The listing builds one solid part. Answer for the finished solid, in the listing's coordinates (mm). Give positions to 0.01 mm unless a question says otherwise; leave off trailing zeros. Write each loop counter-clockwise with the first axis right and the second up, starting at its lowest first coordinate (ties: lowest second). Pieces come first, ordered by that corner, then holes. Notation, with made-up numbers: (-9.5, -25) - (43.5, -25) arc R19 ccw to (43.5, -3) - close; hole circle Ø9 at (-37, -17). An arc over 180 degrees is marked (long way). One line per question, with ' | ' between items. Start each with the question number.
1. A cutting plane is placed at C-C (y = 1.55). Determine the outline of the cut face in (x, z).
2. A cutting plane is placed at D-D (x = 124). Determine the outline of the cut face in (y, z).
3. A cutting plane is placed at A-A (z = -78). Determine the outline of the cut face in (x, y).
4. Find the intervals of material crossed by L1, parallel to X at y = 2.55, z = 17.5; L2, parallel to X at y = 2.65, z = -17.5; L3, parallel to X at y = 1.8, z = 14, in increasing order. Write a range as from..to.
5. Given P1, Ø4, axis at x = -130.89, z = -17.5, coming from the -Y side; P2, Ø0.9, axis at y = 1.5, z = -78, coming from the -X side; P3, Ø1, axis at x = -99, y = 1, coming from the +Z side, each flat-ended and moving along its own axis, determine where each tip first touches the part or whether it passes through.
6. A cutting plane is placed at B-B (x = 13). Determine the outline of the cut face in (y, z), then the cut area to 3 significant figures.
```python
from build123d import *

# Parameters (mm, degrees)
SKETCH1_R           = 142.5
BOSS_EXTRUDE1_DEPTH = 3
SKETCH3_R           = 11
CUT_EXTRUDE1_DEPTH  = 10
CIRPATTERN1_COUNT   = 3
CUT_EXTRUDE2_DEPTH  = 10
CUT_EXTRUDE3_DEPTH  = 10
CUT_EXTRUDE6_START  = -10
CUT_EXTRUDE6_DEPTH  = 10
FILLET1_R           = 3
SKETCH7_W           = 9
SKETCH7_H           = 120
CUT_EXTRUDE7_DEPTH  = 10
SKETCH8_R           = 1.75
CUT_EXTRUDE8_DEPTH  = 10
CHAMFER1_SIZE       = 2.2


with BuildPart() as part:
    # Sketch1 → Boss-Extrude1 (new body)
    with BuildSketch(Plane(origin=(0, 0, 0), x_dir=(1, 0, 0), z_dir=(0, 1, 0))):
        with Locations(Location((0, 0, 0), (0, 0, 270))):
            Circle(SKETCH1_R)
    extrude(amount=BOSS_EXTRUDE1_DEPTH)

    # Sketch3 → Cut-Extrude1 (cut)
    with BuildSketch(Plane(origin=(0, 3, 0), x_dir=(1, 0, 0), z_dir=(0, 1, 0))):
        with Locations(Location((0, -26.5, 0), (0, 0, 270))):
            Circle(SKETCH3_R)
    cut_extrude1 = extrude(amount=-CUT_EXTRUDE1_DEPTH, mode=Mode.SUBTRACT)

    # CirPattern1: Cut-Extrude1 ×3 about axis
    cirpattern1_axis = Axis((0, 0, 0), (0, 1, 0))
    for i in range(1, CIRPATTERN1_COUNT):
        add(cut_extrude1.rotate(cirpattern1_axis, i * 360 / CIRPATTERN1_COUNT), mode=Mode.SUBTRACT)

    # Sketch4 → Cut-Extrude2 (cut)
    with BuildSketch(Plane(origin=(0, 3, 0), x_dir=(1, 0, 0), z_dir=(0, 1, 0))):
        with BuildLine():
            Line((-32.475952642, 7.75), (-9.526279442, -32))
            ThreePointArc((-9.526279442, -32), (0, -37.5), (9.526279442, -32))
            Line((9.526279442, -32), (32.475952642, 7.75))
            ThreePointArc((32.475952642, 7.75), (32.475952642, 18.75), (22.9496732, 24.25))
            Line((22.9496732, 24.25), (-22.9496732, 24.25))
            ThreePointArc((-22.9496732, 24.25), (-32.475952642, 18.75), (-32.475952642, 7.75))
        make_face()
    extrude(amount=-CUT_EXTRUDE2_DEPTH, mode=Mode.SUBTRACT)

    # Sketch5 → Cut-Extrude3 (cut)
    with BuildSketch(Plane(origin=(0, 3, 0), x_dir=(1, 0, 0), z_dir=(0, 1, 0))):
        with BuildLine():
            Line((-5, 45), (-5, 95))
            ThreePointArc((-5, 95), (0, 100), (5, 95))
            Line((5, 95), (5, 45))
            ThreePointArc((5, 45), (0, 40), (-5, 45))
        make_face()
    extrude(amount=-CUT_EXTRUDE3_DEPTH, mode=Mode.SUBTRACT)

    # Sketch6 → Cut-Extrude6 (cut)
    with BuildSketch(Plane(origin=(0, 3, 0), x_dir=(1, 0, 0), z_dir=(0, 1, 0)).offset(CUT_EXTRUDE6_START)):
        with BuildLine():
            Line((89.596317401, -110.809520837), (82.482737092, -103.695940527))
            ThreePointArc((82.482737092, -103.695940527), (93.691648507, -93.691648507), (103.695940527, -82.482737092))
            Line((103.695940527, -82.482737092), (110.809520837, -89.596317401))
            ThreePointArc((110.809520837, -89.596317401), (100.762716319, -100.762716319), (89.596317401, -110.809520837))
        make_face()
    extrude(amount=CUT_EXTRUDE6_DEPTH, mode=Mode.SUBTRACT)

    # Fillet1
    fillet1_edges = [part.edges().sort_by_distance(p)[0] for p in [
        (82.482737092, 1.5, 103.695940527),
        (103.695940527, 1.5, 82.482737092),
        (110.809520837, 1.5, 89.596317401),
        (89.596317401, 1.5, 110.809520837),
    ]]
    fillet(fillet1_edges, radius=FILLET1_R)

    # Sketch7 → Cut-Extrude7 (cut)
    with BuildSketch(Plane(origin=(0, 3, 0), x_dir=(1, 0, 0), z_dir=(0, 1, 0))):
        with Locations((-142.5, 0)):
            Rectangle(SKETCH7_W, SKETCH7_H)
    extrude(amount=-CUT_EXTRUDE7_DEPTH, mode=Mode.SUBTRACT)

    # Sketch8 → Cut-Extrude8 (cut)
    with BuildSketch(Plane(origin=(0, 3, 0), x_dir=(1, 0, 0), z_dir=(0, 1, 0))):
        with Locations(Location((-130.892369907, 17.5, 0), (0, 0, 270))):
            Circle(SKETCH8_R)
        with Locations(Location((-100.892369907, 17.5, 0), (0, 0, 270))):
            Circle(SKETCH8_R)
        with Locations(Location((-130.892369907, -17.5, 0), (0, 0, 270))):
            Circle(SKETCH8_R)
        with Locations(Location((-100.892369907, -17.5, 0), (0, 0, 270))):
            Circle(SKETCH8_R)
    extrude(amount=-CUT_EXTRUDE8_DEPTH, mode=Mode.SUBTRACT)

    # Chamfer1
    chamfer1_edges = [part.edges().sort_by_distance(p)[0] for p in [
        (-130.892369907, 0, -19.25),
        (-100.892369907, 0, -19.25),
        (-130.892369907, 0, 15.75),
        (-100.892369907, 0, 15.75),
    ]]
    chamfer(chamfer1_edges, length=CHAMFER1_SIZE)


solid = part.part
```
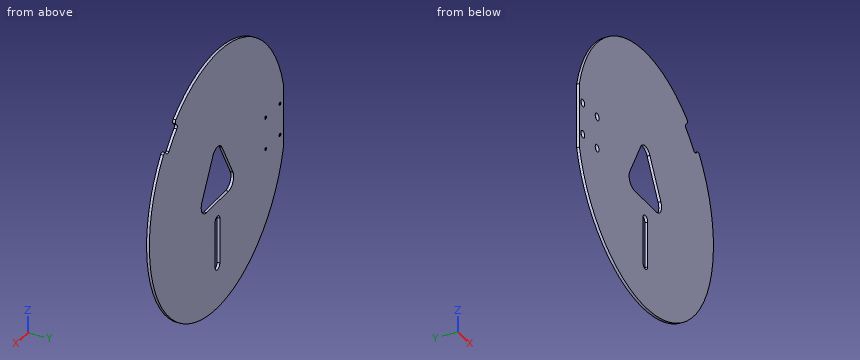
Determined:
1) outline: (-138, -35.53) arc R142.5 ccw (long way) to (112.92, 86.92) arc R3 ccw to (108.42, 87.21) - (106.04, 84.83) arc R3 cw to (101.62, 85.03) arc R132.5 ccw to (85.03, 101.62) arc R3 cw to (84.83, 106.04) - (87.21, 108.42) arc R3 ccw to (86.92, 112.92) arc R142.5 ccw to (-138, 35.53) - close; hole circle Ø4.8 at (-130.89, -17.5); hole circle Ø4.8 at (-130.89, 17.5); hole circle Ø4.8 at (-100.89, -17.5); hole circle Ø4.8 at (-100.89, 17.5); hole (-32.48, -7.75) arc R11 ccw to (-22.95, -24.25) - (22.95, -24.25) arc R11 ccw to (32.48, -7.75) - (9.53, 32) arc R11 ccw to (-9.53, 32) - close; hole (-5, -95) arc R5 ccw to (5, -95) - (5, -45) arc R5 ccw to (-5, -45) - close
2) outline: (0, -70.22) - (3, -70.22) - (3, 70.22) - (0, 70.22) - close
3) outline: (-119.26, 0) - (-5, 0) - (-5, 3) - (-119.26, 3) - close; (5, 0) - (119.26, 0) - (119.26, 3) - (5, 3) - close
4) L1: -138..-132.64, -129.14..-102.64, -99.14..-17.9, 17.9..141.42 | L2: -138..-132.64, -129.14..-102.64, -99.14..-33.1, 33.1..141.42 | L3: -138..-19.92, 19.92..141.81
5) P1: y = 1.95 | P2: x = -119.55 | P3: z = 102.98
6) outline: (0, -141.91) - (3, -141.91) - (3, -24.25) - (0, -24.25) - close; (0, 25.98) - (3, 25.98) - (3, 141.91) - (0, 141.91) - close | area: 701 mm2
